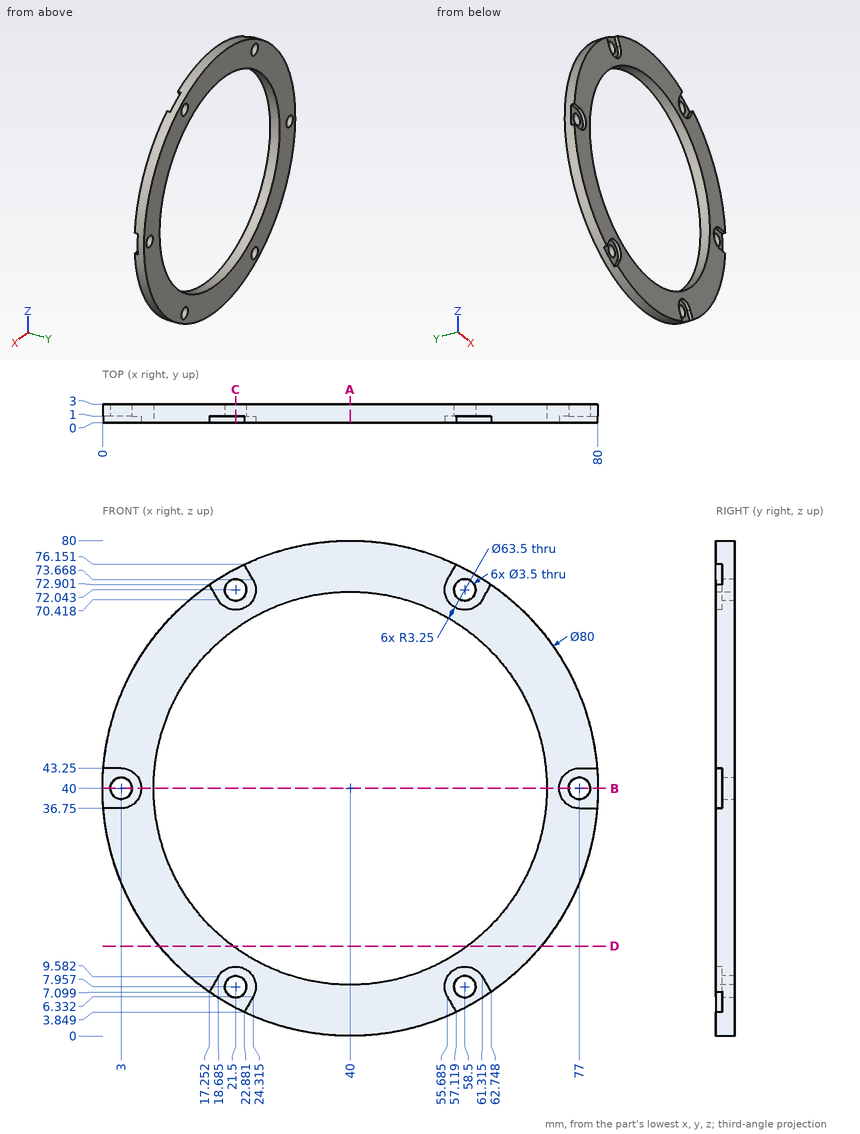
Input: dimensioned drawing with shaded views. Units: mm. Origin: part minimum x, y, z. Round coordinates to 2 decimals unless told otherwise and drop trailing zeros. Loops run counter-clockwise (first coordinate to the right, second up) from the corner with the lowest first, then second, coordinate; pieces in that order, holes last.
1) Section query D-D on z = 14.5. Return the cut outline in (x, y) (1 decimal).
Ans:
outline: (9.2, 0) - (21.1, 0) - (21.1, 3) - (9.2, 3) - close; (58.9, 0) - (70.8, 0) - (70.8, 3) - (58.9, 3) - close
2) Section query B-B on z = 40. Return the cut outline in (x, y), plus the area to 3 significant figures.
Ans:
outline: (0, 1) - (1.25, 1) - (1.25, 3) - (0, 3) - close; (4.75, 1) - (6.25, 1) - (6.25, 0) - (8.25, 0) - (8.25, 3) - (4.75, 3) - close; (71.75, 0) - (73.75, 0) - (73.75, 1) - (75.25, 1) - (75.25, 3) - (71.75, 3) - close; (78.75, 1) - (80, 1) - (80, 3) - (78.75, 3) - close
area: 23.0 mm2
3) Material intervals for line 1 (X direction, y = 2.25, z = 40); line 2 (Z direction, x = 20, y = 2.2) (1 decimal); line 3 (Y direction, x = 57, z = 73), sorted ascending.
Ans:
line 1: x = 0 to 1.25, 4.75 to 8.25, 71.75 to 75.25, 78.75 to 80
line 2: z = 5.4 to 7.1, 8.9 to 15.3, 64.7 to 71.1, 72.9 to 74.6
line 3: y = 1 to 3
4) Section query A-A on x = 40. Return the cut outline in (y, z), plus the area to 3 significant figures.
Ans:
outline: (0, 0) - (3, 0) - (3, 8.25) - (0, 8.25) - close; (0, 71.75) - (3, 71.75) - (3, 80) - (0, 80) - close
area: 49.5 mm2
5) Section query C-C on x = 21.5. Return the cut outline in (y, z) (1 decimal).
Ans:
outline: (0, 11.2) - (1, 11.2) - (1, 9.7) - (3, 9.7) - (3, 14.2) - (0, 14.2) - close; (0, 65.8) - (3, 65.8) - (3, 70.3) - (1, 70.3) - (1, 68.8) - (0, 68.8) - close; (1, 4.5) - (3, 4.5) - (3, 6.2) - (1, 6.2) - close; (1, 73.8) - (3, 73.8) - (3, 75.5) - (1, 75.5) - close
6) Pin query (flat end, axial travel): pin 1 (2 mm diameter, centred on x = 61, z = 71.5, fed in from -Y); pin 2 (3 mm diameter, centred on x = 4, z = 41, fed in from -Y); pin 3 (3 mm diameter, centred on x = 21.5, z = 7.96, fed in from +Y); pin 4 (1.5 mm diameter, centred on x = 23.5, y = 1, fed in from -Z). Return the tip coordinate at first contact, or that it passes through.
Ans:
pin 1: stops at y = 0
pin 2: stops at y = 1
pin 3: passes through
pin 4: stops at z = 3.23
